Input: part model. Units: mm. Frame: model coordinates. A direction names the side the tool comes from. Give positions to 0.01 mm unless a question says otherwise; leave off trailing zeros. Write each loop counter-clockwise with the first axis right and the second up, starting at its lowest first coordinate (ties: lowest second). Pieces come first, ordered by that corner, then holes. Notation, with made-up numbers: (70, -34) -> (90, -34) arc R11 cw to (90, -20) -> close; hole circle Ø2 at (-33, 50). An arc over 180 degrees is marked (long way). Return JSON: item names as keys, results as strings. Group by question number.
Item 1: Pin query (flat end, axial travel): P1, Ø1.5, axis at x = 21, z = 53.5, coming from the -Y side; P2, Ø1.5, axis at x = 17, z = 50, coming from the -Y side; P3, Ø8, axis at x = 108, y = 59, coming from the +Z side; P4, Ø15, axis at y = 37.5, z = 50, coming from the +X side. Return the tip coordinate at first contact, or that it passes through.
Item 2: Line query: line 1 (X direction, y = 12, z = 32); line 2 (Z direction, x = 103.5, y = 31.5); line 3 (X direction, y = 36.5, z = -7.5). Output: solid intervals per line, ascending. Write a range as [from, to].
Item 3: Section B-B, the plane z = 53.5. Return loops of the section in (x, y), then the cut area to 3 significant figures.
Item 4: Section D-D, the plane z = 5. Return loops of the section in (x, y).
Item 5: Section C-C, the plane x = 90. Return loops of the section in (y, z), then the cut area to 3 significant figures.
Item 6: Mould query, pull axis X, two halves, no side actions, for faces 5 (the face through (22, 46, 39)), 6 (the face through (0, 38, 29)), 7 (the face through (114.846, 36.95, 37.512)). Classes: released by +X, released by -X, zero draft, split by the parting line, or undercut.
Item 7: Set-up query: faces 1 (the face through (63, 38, 3)), 2 (the face through (67.56, 72.2, -14.79)), 3 (the face through (11.15, 8.48, 44.52)), 4 (the face through (44, 46, 25)). Return all of +Z, -Z, +X, -X, +Y, -Y with unobstructed straight access to the full face (end or side cutting, diameter ignored); none if empty.
Item 8: Section A-A, the plane y = 41.5. Return loops of the section in (x, z), then the cut area to 3 significant figures.
from build123d import *

# Parameters (mm, degrees)
BASE_PLATE_SKETCH_W  = 126
BASE_PLATE_SKETCH_H  = 75
BASE_PLATE_DEPTH     = 25
LUG_1_DEPTH          = 22
LUG_START            = -22
LUG_2_DEPTH          = 22
CENTRE_BORE_SKETCH_R = 20
CENTRE_BORE_40_DEPTH = 22
REAR_BOSS_SKETCH_R   = 35
REAR_BOSS_70_DEPTH   = 30
LUG_HOLE_1_SKETCH_R  = 12.5
LUG_HOLE_1_25_DEPTH  = 22
LUG_HOLE_2_SKETCH_R  = 12.5
LUG_HOLE_2_25_DEPTH  = 22


with BuildPart() as part:
    # Base Plate Sketch → Base Plate (new body)
    with BuildSketch(Plane.XY):
        with Locations((63, 37.5)):
            Rectangle(BASE_PLATE_SKETCH_W, BASE_PLATE_SKETCH_H)
    extrude(amount=BASE_PLATE_DEPTH)

    # Lug 1 Sketch → Lug 1 (add)
    with BuildSketch(Plane(origin=(126, 0, 0), x_dir=(0, 0, -1), z_dir=(1, 0, 0))):
        with BuildLine():
            Line((-25, 75), (-25, 0))
            Line((-25, 0), (-63.918991375, 16.733159145))
            ThreePointArc((-63.918991375, 16.733159145), (-75, 37.5), (-63.918991375, 58.266840855))
            Line((-63.918991375, 58.266840855), (-25, 75))
        make_face()
    extrude(amount=-LUG_1_DEPTH)

    # Lug 2 Sketch → Lug 2 (add)
    with BuildSketch(Plane.ZY.offset(LUG_START)):
        with BuildLine():
            Line((25, 75), (25, 0))
            Line((25, 0), (64.599836332, 17.206040823))
            ThreePointArc((64.599836332, 17.206040823), (74.996563929, 37.914477664), (63.918991375, 58.266840855))
            Line((63.918991375, 58.266840855), (25, 75))
        make_face()
    extrude(amount=LUG_2_DEPTH)

    # Centre Bore Sketch → Centre Bore Ø40 (cut)
    with BuildSketch(Plane.XY.offset(25)):
        with Locations((63, 37.736440839)):
            Circle(CENTRE_BORE_SKETCH_R)
    extrude(amount=-CENTRE_BORE_40_DEPTH, mode=Mode.SUBTRACT)

    # Rear Boss Sketch → Rear Boss Ø70 (add)
    with BuildSketch(Plane(origin=(0, 0, 0), x_dir=(-1, 0, 0), z_dir=(0, 0, -1))):
        with Locations((-63, 37.5)):
            Circle(REAR_BOSS_SKETCH_R)
    extrude(amount=REAR_BOSS_70_DEPTH)

    # Lug Hole 1 Sketch → Lug Hole 1 Ø25 (cut)
    with BuildSketch(Plane.ZY):
        with Locations((50, 37.5)):
            Circle(LUG_HOLE_1_SKETCH_R)
    extrude(amount=-LUG_HOLE_1_25_DEPTH, mode=Mode.SUBTRACT)

    # Lug Hole 2 Sketch → Lug Hole 2 Ø25 (cut)
    with BuildSketch(Plane(origin=(126, 0, 0), x_dir=(0, 0, -1), z_dir=(1, 0, 0)).offset(LUG_START)):
        with Locations(Location((-50, 37.5, 0), (0, 0, 180))):
            Circle(LUG_HOLE_2_SKETCH_R)
    extrude(amount=LUG_HOLE_2_25_DEPTH, mode=Mode.SUBTRACT)


solid = part.part
Answer below:
{
 "1": {"P1": "stops at y = 12.06", "P2": "stops at y = 10.54", "P3": "stops at z = 67.85", "P4": "passes through"},
 "2": {"line 1": "x = [0, 22], [104, 126]", "line 2": "z = [0, 25]", "line 3": "x = [28.01, 97.99]"},
 "3": {"outline": "(0, 12.38) -> (22, 12.38) -> (22, 25.5) -> (0, 25.5) -> close; (0, 49.5) -> (22, 49.5) -> (22, 62.75) -> (0, 62.75) -> close; (104, 12.25) -> (126, 12.25) -> (126, 25.5) -> (104, 25.5) -> close; (104, 49.5) -> (126, 49.5) -> (126, 62.75) -> (104, 62.75) -> close", "area": "1,160 mm2"},
 "4": {"outline": "(0, 0) -> (126, 0) -> (126, 75) -> (0, 75) -> close; hole circle Ø40 at (63, 37.74)"},
 "5": {"outline": "(0, 0) -> (15.23, 0) -> (15.23, -30) -> (59.77, -30) -> (59.77, 0) -> (75, 0) -> (75, 25) -> (0, 25) -> close", "area": "3,210 mm2"},
 "6": {"face 5": "undercut", "face 6": "released by -X", "face 7": "zero draft"},
 "7": {"face 1": "+Z", "face 2": "-Z", "face 3": "+Z, -X, -Y", "face 4": "+Z, +Y, -Y"},
 "8": {"outline": "(0, 0) -> (28.23, 0) -> (28.23, -30) -> (97.77, -30) -> (97.77, 0) -> (126, 0) -> (126, 38.16) -> (104, 38.16) -> (104, 25) -> (82.64, 25) -> (82.64, 3) -> (43.36, 3) -> (43.36, 25) -> (22, 25) -> (22, 38.16) -> (0, 38.16) -> close; (0, 61.84) -> (22, 61.84) -> (22, 74.68) -> (0, 74.68) -> close; (104, 61.84) -> (126, 61.84) -> (126, 74.68) -> (104, 74.68) -> close", "area": "5,520 mm2"}
}
